For this review, use the dimensioned drawing (mm, ordinates from the lowest corner) and the shaded views. A direction names the side the tool comes from. Give positions to 0.01 mm unless a question says otherwise; leave off trailing zeros. Order: outer loops, then holes, each group sorted by start corner. A loop starts at its lowest first (then second) coordinate and runs counter-clockwise, first axis right, second up.
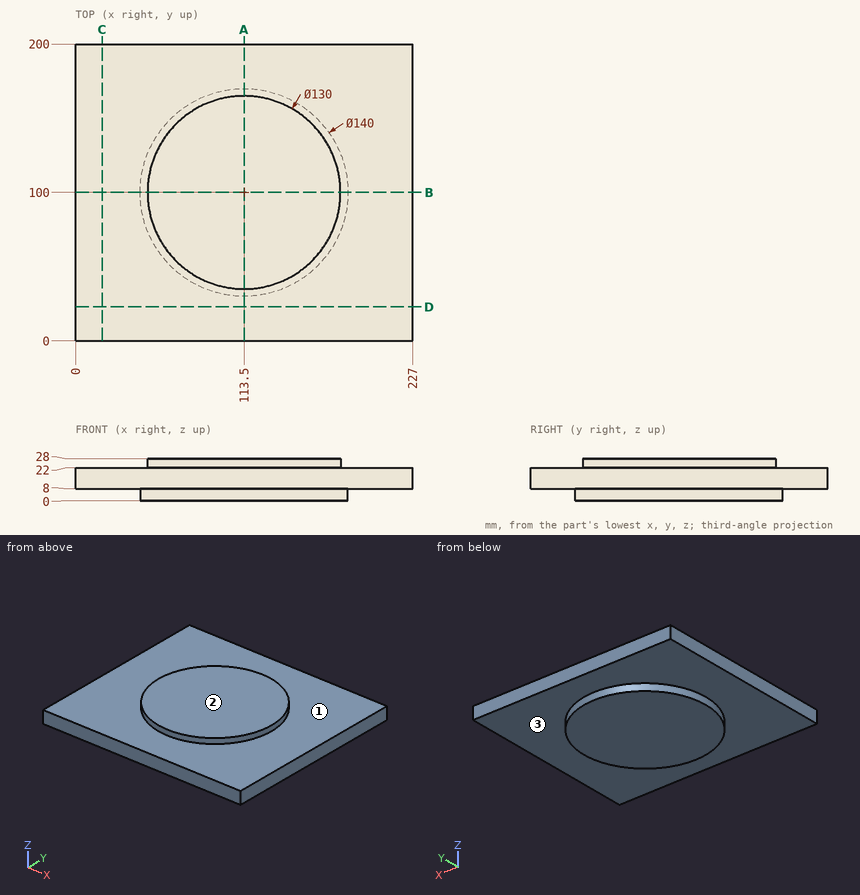
1. Take a section at C-C (x = 18). State the section outline as (y, z) points, then the cut area to 3 significant figures.
Recorded:
outline: (0, 8) - (200, 8) - (200, 22) - (0, 22) - close
area: 2,800 mm2
2. For line 1 along Z through (x, y) = (37, 187); line 2 along X through (y, z) = (38, 4.75); line 3 along X through (y, z) = (110.5, 5), list the stretches that pass through material, from the lowest coordinate up.
Recorded:
line 1: z = 8 to 22
line 2: x = 81 to 146
line 3: x = 44.29 to 182.71
3. Take a section at D-D (y = 23). State the section outline as (x, z) points.
Recorded:
outline: (0, 8) - (227, 8) - (227, 22) - (0, 22) - close
4. For pin 1 (1 mm diameter, centred on y = 46.5, z = 3.5, fed in from -X); pin 2 (4 mm diameter, centred on y = 21.5, z = 19.5, fed in from -X); pin 3 (2 mm diameter, centred on y = 61, z = 6, fed in from -X), all flat-tipped, find the tip position at first contact; note any pin that passes through.
Recorded:
pin 1: stops at x = 67.77
pin 2: stops at x = 0
pin 3: stops at x = 54.71
5. Take a section at A-A (x = 113.5). State the section outline as (y, z) points.
Recorded:
outline: (0, 8) - (30, 8) - (30, 0) - (170, 0) - (170, 8) - (200, 8) - (200, 22) - (165, 22) - (165, 28) - (35, 28) - (35, 22) - (0, 22) - close
6. Take a section at B-B (y = 100). State the section outline as (x, z) points.
Recorded:
outline: (0, 8) - (43.5, 8) - (43.5, 0) - (183.5, 0) - (183.5, 8) - (227, 8) - (227, 22) - (178.5, 22) - (178.5, 28) - (48.5, 28) - (48.5, 22) - (0, 22) - close
7. Machinability: for the marked faces 1, 2 and 3, which of the approach directions +Z, -Z, +X, -X, +Y, -Y give a long, thin tool a straight path to every point of the face, cutting with its end or side? Answer none if there is none.
Recorded:
face 1: +Z
face 2: +Z, +X, -X, +Y, -Y
face 3: -Z
